from build123d import *

# Parameters (mm, degrees)
SKETCH1_W           = 1170
SKETCH1_H           = 740
BOSS_EXTRUDE1_DEPTH = 7.5
SKETCH2_W           = 245
SKETCH2_H           = 190
SKETCH2_W_2         = 240
CUT_EXTRUDE1_DEPTH  = 108


with BuildPart() as part:
    # Sketch1 → Boss-Extrude1 (new, symmetric)
    with BuildSketch(Plane(origin=(0, 0, 0), x_dir=(0, 0, -1), z_dir=(1, 0, 0))):
        Rectangle(SKETCH1_W, SKETCH1_H)
    extrude(amount=BOSS_EXTRUDE1_DEPTH, both=True)

    # Sketch2 → Cut-Extrude1 (cut)
    with BuildSketch(Plane(origin=(7.5, 0, 0), x_dir=(0, 0, -1), z_dir=(1, 0, 0))):
        with Locations((-422.5, 235)):
            Rectangle(SKETCH2_W, SKETCH2_H)
        with Locations((-422.5, 0)):
            Rectangle(SKETCH2_W, SKETCH2_H)
        with Locations((-140, 0)):
            Rectangle(SKETCH2_W_2, SKETCH2_H)
        with Locations((-140, 235)):
            Rectangle(SKETCH2_W_2, SKETCH2_H)
        with Locations((-422.5, -235)):
            Rectangle(SKETCH2_W, SKETCH2_H)
        with Locations((-140, -235)):
            Rectangle(SKETCH2_W_2, SKETCH2_H)
    cut_extrude1 = extrude(amount=-CUT_EXTRUDE1_DEPTH, mode=Mode.SUBTRACT)

    # Mirror1: Cut-Extrude1 across plane
    add(cut_extrude1.mirror(Plane.XY), mode=Mode.SUBTRACT)


solid = part.part
Here's how the part is built. I have some questions about the finished solid (model axes, mm). Coordinates: 2 decimals unless noted, no trailing zeros. Order: outer loops, then holes, each group sorted by start corner. A loop starts at its lowest first (then second) coordinate and runs counter-clockwise, first axis right, second up. Notation, with made-up numbers: (46.5, -27.75) - (50.5, -27.75) arc R34 cw to (50.5, 2.25) - close; hole circle Ø5 at (9.5, 35.25). An arc over 180 degrees is marked (long way). Use CSV: the item, a comma, the result in double quotes. Start each with the question number.
1. Suppose I cut it at A-A on z = 148.5. List the corners of the cut face in (x, y) for me, then the cut area to 3 significant figures.
2. Please list where these lines run through material, in increasing order: line 1 (Y direction, x = 2.5, z = 130.5); line 2 (Z direction, x = 6.5, y = 176). Write a range as from..to.
3. Suppose I cut it at B-B on y = -307. List the corners of the cut face in (x, z) for me, then the cut area to 3 significant figures.
4. Suppose I cut it at C-C on x = -5. Give the number of separate pieces and of enclosed holes in the cut face, then the cut area to 3 significant figures.
Output:
1,outline,"(-7.5, -370) - (7.5, -370) - (7.5, -330) - (-7.5, -330) - close; (-7.5, -140) - (7.5, -140) - (7.5, -95) - (-7.5, -95) - close; (-7.5, 95) - (7.5, 95) - (7.5, 140) - (-7.5, 140) - close; (-7.5, 330) - (7.5, 330) - (7.5, 370) - (-7.5, 370) - close"
1,area,"2,550 mm2"
2,line 1,"y = -370..-330, -140..-95, 95..140, 330..370"
2,line 2,"z = -585..-545, -300..-260, -20..20, 260..300, 545..585"
3,outline,"(-7.5, -585) - (7.5, -585) - (7.5, -545) - (-7.5, -545) - close; (-7.5, -300) - (7.5, -300) - (7.5, -260) - (-7.5, -260) - close; (-7.5, -20) - (7.5, -20) - (7.5, 20) - (-7.5, 20) - close; (-7.5, 260) - (7.5, 260) - (7.5, 300) - (-7.5, 300) - close; (-7.5, 545) - (7.5, 545) - (7.5, 585) - (-7.5, 585) - close"
3,area,"3,000 mm2"
4,separate pieces,"1"
4,enclosed holes,"12"
4,area,"313,000 mm2"
